from build123d import *

# Parameters (mm, degrees)
SKETCH1_W             = 33
SKETCH1_H             = 15
BOSS_EXTRUDE1_DEPTH   = 10
SKETCH2_W             = 23
SKETCH2_H             = 10
CUT_EXTRUDE1_DEPTH    = 20
M4_TAPPED_HOLE1_D     = 3.3
M4_TAPPED_HOLE1_DEPTH = 10.1
M4_TAPPED_HOLE1_TIP   = 0.991420021
CHAMFER1_SIZE         = 0.5
SKETCH6_R             = 3.5
CUT_EXTRUDE3_DEPTH    = 2.5
SKETCH7_R             = 1.6
CUT_EXTRUDE4_DEPTH    = 3
SKETCH8_R             = 2.05
CUT_EXTRUDE5_DEPTH    = 10


with BuildPart() as part:
    # Sketch1 → Boss-Extrude1 (new body)
    with BuildSketch(Plane.XY):
        Rectangle(SKETCH1_W, SKETCH1_H)
    extrude(amount=BOSS_EXTRUDE1_DEPTH)

    # Sketch2 → Cut-Extrude1 (cut)
    with BuildSketch(Plane.XY.offset(10)):
        with Locations((5, -2.5)):
            Rectangle(SKETCH2_W, SKETCH2_H)
    extrude(amount=-CUT_EXTRUDE1_DEPTH, mode=Mode.SUBTRACT)

    # M4 Tapped Hole1
    with Locations(Plane(origin=(0, -7.5, 0), x_dir=(-1, 0, 0), z_dir=(0, -1, 0))):
        with Locations((11.5, -5)):
            Hole(M4_TAPPED_HOLE1_D / 2, depth=M4_TAPPED_HOLE1_DEPTH)
            with Locations((0, 0, -(M4_TAPPED_HOLE1_DEPTH + M4_TAPPED_HOLE1_TIP / 2))):  # 118° drill point
                Cone(0, M4_TAPPED_HOLE1_D / 2, M4_TAPPED_HOLE1_TIP, mode=Mode.SUBTRACT)

    # Chamfer1
    chamfer1_edges = [part.edges().sort_by_distance(p)[0] for p in [
        (-16.5, 0, 10),
        (-11.5, -7.5, 10),
        (5, 2.5, 0),
        (-6.5, -2.5, 0),
        (16.5, 2.5, 5),
        (-6.5, -7.5, 5),
        (5, 2.5, 10),
        (-6.5, -2.5, 10),
        (-11.5, -7.5, 0),
        (-16.5, 0, 0),
        (0, 7.5, 0),
        (0, 7.5, 10),
        (-16.5, -7.5, 5),
        (-16.5, 7.5, 5),
        (16.5, 7.5, 5),
    ]]
    chamfer(chamfer1_edges, length=CHAMFER1_SIZE)

    # Sketch6 → Cut-Extrude3 (cut)
    with BuildSketch(Plane(origin=(0, 7.5, 0), x_dir=(1, 0, 0), z_dir=(0, 1, 0))):
        with Locations(Location((3.5, -5, 0), (0, 0, 270))):
            Circle(SKETCH6_R)
    extrude(amount=-CUT_EXTRUDE3_DEPTH, mode=Mode.SUBTRACT)

    # Sketch7 → Cut-Extrude4 (cut)
    with BuildSketch(Plane(origin=(0, 0, 0), x_dir=(-1, 0, 0), z_dir=(0, 0, -1))):
        with Locations((-13.5, 5)):
            Circle(SKETCH7_R)
    cut_extrude4 = extrude(amount=-CUT_EXTRUDE4_DEPTH, mode=Mode.SUBTRACT)

    # Mirror1: Cut-Extrude4 across plane
    add(cut_extrude4.mirror(Plane(origin=(0, 0, 5), x_dir=(1, 0, 0), z_dir=(0, 0, -1))), mode=Mode.SUBTRACT)

    # Sketch8 → Cut-Extrude5 (cut)
    with BuildSketch(Plane(origin=(0, 5, 0), x_dir=(1, 0, 0), z_dir=(0, 1, 0))):
        with Locations(Location((3.5, -5, 0), (0, 0, 270))):
            Circle(SKETCH8_R)
    extrude(amount=-CUT_EXTRUDE5_DEPTH, mode=Mode.SUBTRACT)


solid = part.part
Model file for the job. Use its own axes, mm. A direction names the side the tool comes from. Give positions to 0.01 mm unless a question says otherwise; leave off trailing zeros. Order: outer loops, then holes, each group sorted by start corner. A loop starts at its lowest first (then second) coordinate and runs counter-clockwise, first axis right, second up. Notation, with made-up numbers: M 65,72 L 96,72 A18 ccw 96,89 Z; hole C 59,-36.75 d3. An arc over 180 degrees is marked long. Write item = value, one per line.
Q1. Two-plate mould, pull along Y, no slides. Class faces 4 (the flat face through (-3.6, 3.2, 10)), 5 (the cylindrical face through (15.1, 5.07, 8.52)), 6 (the flat face through (5, 2.5, 3)): pulls with the +Y half, pulls with the -Y half, needs draft (parallel to the pull), parting line crosses it, or undercut.
Derived:
face_4 = needs draft
face_5 = undercut
face_6 = pulls with the -Y half
Q2. Flat gauge pins, fed straight in: pin 1 (3 mm diameter, centred on y = -0.5, z = 2, fed in from +X); pin 2 (3 mm diameter, centred on x = 4.5, z = 7.5, fed in from -Y); pin 3 (1 mm diameter, centred on x = 14, y = 5, fed in from +Z). Where does each tip first touch, or does it go through?
Derived:
pin_1 = -6.5
pin_2 = 2.5
pin_3 = 7
Q3. Cut at C-C, the plane x = 13.5. List the corners of the cut face in (y, z), then the cut area to 3 significant figures.
Derived:
outline = M 2.5,0.5 L 3,0 L 3.4,0 L 3.4,3 L 6.6,3 L 6.6,0 L 7,0 L 7.5,0.5 L 7.5,9.5 L 7,10 L 6.6,10 L 6.6,7 L 3.4,7 L 3.4,10 L 3,10 L 2.5,9.5 Z
area = 30.3 mm2
Q4. Tool access for faces 1 (the flat face through (14, 5, 3)), 2 (the flat face through (-6.5, -2, 5)), 3 (the cylindrical face through (-9.976, -2.379, 5.632)): list every direction of +Z, -Z, +X, -X, +Y, -Y with a clear straight run to the whole face (end or side of a thin tool).
Derived:
face_1 = -Z
face_2 = +Z, -Z, +X, -Y
face_3 = -Y
Q5. Drill centre lines: line 1 (X direction, y = -0.75, z = 5); line 2 (Y direction, x = 13.5, z = 1.55); line 3 (X direction, y = 4.5, z = 5). Where is each one in solid material? Low to high. Write a range as [from, to].
Derived:
line_1 = [-16.5, -13.15], [-9.85, -6.5]
line_2 = [2.5, 3.4], [6.6, 7.5]
line_3 = [-16.5, 1.45], [5.55, 16.5]
Q6. Cut at A-A, the plane x = 3.5. List the corners of the cut face in (y, z), then the cut area to 4 significant figures.
Derived:
outline = M 2.5,0.5 L 3,0 L 7,0 L 7.5,0.5 L 7.5,1.5 L 5,1.5 L 5,2.95 L 2.5,2.95 Z; M 2.5,7.05 L 5,7.05 L 5,8.5 L 7.5,8.5 L 7.5,9.5 L 7,10 L 3,10 L 2.5,9.5 Z
area = 21.75 mm2
Q7. Cut at B-B, the plane y = -3.25. List the corners of the cut face in (x, z).
Derived:
outline = M -16.5,0.5 L -16,0 L -7,0 L -6.5,0.5 L -6.5,9.5 L -7,10 L -16,10 L -16.5,9.5 Z; hole C -11.5,5 d3.3
